Design review of the part built by this model. Coordinates are the model's own, in mm. Face numbers are marked on the shaded views. A direction names the side the tool comes from. Coordinates: 2 decimals unless noted, no trailing zeros. Order: outer loops, then holes, each group sorted by start corner. A loop starts at its lowest first (then second) coordinate and runs counter-clockwise, first axis right, second up. Notation, with made-up numbers: (22, -8.5) - (63, -8.5) arc R13 cw to (63, 9.5) - close; hole circle Ø11 at (57, -8.5). An arc over 180 degrees is marked (long way). Write each question's results on one line, items separated by ' | '. Start each with the question number.
```python
from build123d import *

# Parameters (mm, degrees)
BOSS_EXTRUDE1_DEPTH = 3.6
SKETCH2_R           = 31.666666667
CUT_EXTRUDE1_DEPTH  = 1
SKETCH4_R           = 5.5
CUT_EXTRUDE2_DEPTH  = 78.385241649


with BuildPart() as part:
    # Sketch1 → Boss-Extrude1 (new body)
    with BuildSketch(Plane(origin=(0, 0, 0), x_dir=(1, 0, 0), z_dir=(0, 1, 0))):
        with BuildLine():
            Line((-37, 50), (37, 50))
            ThreePointArc((37, 50), (51.142135624, 44.142135624), (57, 30))
            Line((57, 30), (57, -30))
            ThreePointArc((57, -30), (51.142135624, -44.142135624), (37, -50))
            Line((37, -50), (-37, -50))
            ThreePointArc((-37, -50), (-51.142135624, -44.142135624), (-57, -30))
            Line((-57, -30), (-57, 30))
            ThreePointArc((-57, 30), (-51.142135624, 44.142135624), (-37, 50))
        make_face()
    extrude(amount=-BOSS_EXTRUDE1_DEPTH)

    # Sketch2 → Cut-Extrude1 (cut)
    with BuildSketch(Plane(origin=(0, 0, 0), x_dir=(1, 0, 0), z_dir=(0, 1, 0))):
        with Locations(Location((0, 0, 0), (0, 0, 270))):
            Circle(SKETCH2_R)
    extrude(amount=-CUT_EXTRUDE1_DEPTH, mode=Mode.SUBTRACT)

    # Sketch3 → Revolve1 (revolve)
    with BuildSketch(Plane.XY, mode=Mode.PRIVATE) as revolve1_sk:
        with BuildLine():
            Line((0, -3.6), (38, -3.6))
            Line((38, -3.6), (31.599978616, -14.488457433))
            ThreePointArc((31.599978616, -14.488457433), (30.869015975, -15.210931287), (29.875767483, -15.475))
            Line((29.875767483, -15.475), (0, -15.475))
            Line((0, -15.475), (0, -3.6))
        make_face()
    revolve(revolve1_sk.sketch.rotate(Axis((0, -15.475, 0), (0, 1, 0)), 270), axis=Axis((0, -15.475, 0), (0, 1, 0)))

    # Sketch4 → Cut-Extrude2 (cut, through all)
    with BuildSketch(Plane(origin=(0, 0, 0), x_dir=(1, 0, 0), z_dir=(0, 1, 0))):
        with Locations(Location((-42, 35.5, 0), (0, 0, 270))):
            Circle(SKETCH4_R)
        with Locations(Location((42, 35.5, 0), (0, 0, 270))):
            Circle(SKETCH4_R)
        with Locations(Location((42, -35.5, 0), (0, 0, 270))):
            Circle(SKETCH4_R)
        with Locations(Location((-42, -35.5, 0), (0, 0, 270))):
            Circle(SKETCH4_R)
    extrude(amount=-CUT_EXTRUDE2_DEPTH, mode=Mode.SUBTRACT)


solid = part.part
```
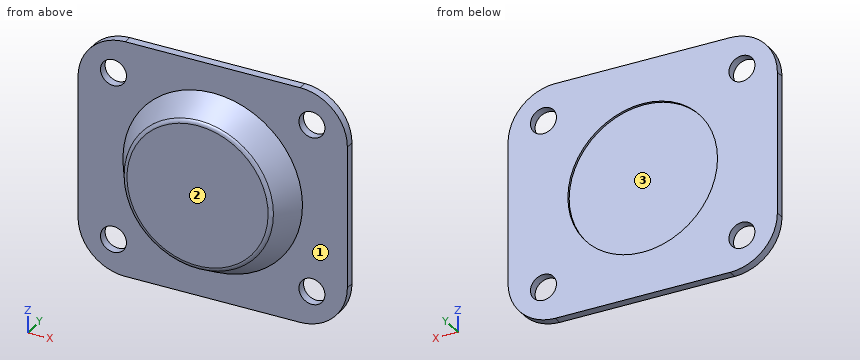
(1) Take a section at C-C (x = 0). State the section outline as (y, z) points (3 decimals), plus the area to 3 significant figures.
(2) Take a section at D-D (z = 35.5). State how many separate pieces and enclosed holes the cut face has, plus the area to 3 significant figures.
(3) Tool access review of the marked faces 1, 2 and 3: name each direction out of +Z, -Z, +X, -X, +Y, -Y from which nothing blocks a thin tool from reaching the whole face with its end or side.
(4) Take a section at A-A (x = -42). State the section outline as (y, z) points, plus the area to 3 significant figures.
(5) Clearance check with flat-ended pins moving along their axes: pin 1 (5 mm diameter, centred on x = -29.5, z = 37, fed in from -Y); pin 2 (2 mm diameter, centred on x = 8, y = -7.5, fed in from -Z); pin 3 (3 mm diameter, centred on y = -6.5, z = 14.5, fed in from +X). State where each tip first meets the part, or that it passes through.
(6) To check wall thickness, follow line 1 along Z through (x, y) = (-40, -3.5); line 2 along X through (y, z) = (-2, 35.5); line 3 along Y through (x, z) = (13, -12) (3 decimals). State the ranges of each line that lie inside material, in increasing order. Write a range as [from, to].
(7) Take a section at B-B (z = 0). State the section outline as (x, y) points (3 decimals).
Worked out:
1) outline: (-15.475, -29.876) arc R2 ccw to (-14.488, -31.6) - (-3.6, -38) - (-3.6, -50) - (0, -50) - (0, -31.667) - (-1, -31.667) - (-1, 31.667) - (0, 31.667) - (0, 50) - (-3.6, 50) - (-3.6, 38) - (-14.488, 31.6) arc R2 ccw to (-15.475, 29.876) - close | area: 1,120 mm^2
2) separate pieces: 3 | enclosed holes: 0 | area: 402 mm^2
3) face 1: -Y | face 2: +Z, -Z, +X, -X, -Y | face 3: +Y
4) outline: (-3.6, -49.36) - (0, -49.36) - (0, -41) - (-3.6, -41) - close; (-3.6, -30) - (0, -30) - (0, 30) - (-3.6, 30) - close; (-3.6, 41) - (0, 41) - (0, 49.36) - (-3.6, 49.36) - close | area: 276 mm^2
5) pin 1: y = -3.6 | pin 2: z = -35.44 | pin 3: x = 34.41
6) line 1: [-49.77, -40.62], [-30.38, 30.38], [40.62, 49.77] | line 2: [-56.23, -47.5], [-36.5, 36.5], [47.5, 56.23] | line 3: [-15.475, -1]
7) outline: (-57, -3.6) - (-38, -3.6) - (-31.6, -14.488) arc R2 ccw to (-29.876, -15.475) - (29.876, -15.475) arc R2 ccw to (31.6, -14.488) - (38, -3.6) - (57, -3.6) - (57, 0) - (31.667, 0) - (31.667, -1) - (-31.667, -1) - (-31.667, 0) - (-57, 0) - close
